Work out the finished part from the listing and answer in its coordinate system (mm). Face numbers are marked on the shaded views. Round coordinates to 2 decimals unless told otherwise and drop trailing zeros. Loops run counter-clockwise (first coordinate to the right, second up) from the corner with the lowest first, then second, coordinate; pieces in that order, holes last. Notation, with made-up numbers: (56, 69) - (106, 69) arc R15 cw to (106, 83) - close; hole circle Ø5 at (12, 31.5). An arc over 180 degrees is marked (long way). Answer as CSV lines item,"result". Start each with the question number.
Q1. Each of these flat-tipped pins is pushed along its axis until it touches: pin 1 Ø5 at (y, z) = (53, 30.5) entering from +X; pin 2 Ø1 at (x, y) = (16.5, 42) entering from +Z; pin 3 Ø3 at (x, z) = (20, 35) entering from +Y; pin 4 Ø3 at (x, z) = (22, -43) entering from -Y. Where does it stop, or does it pass through?
Q2. The mould has two halves that part along Z. Classify the marked faces 1, 2, 3 and 4: +Z half, -Z half, draft (parallel to the pull), parting line (faces both ways), or undercut.
Q3. Straight lines are drawn through the part: L1, parallel to Y at x = 11.25, z = 48.5; L2, parallel to Y at x = 10.25, z = 0; L3, parallel to Y at x = 18.75, z = 48.5. For each, find the intervals that lie inside material, in ascending order. Write a range as [from, to].
Q4. Section B-B on y = 0 is taken. Write down the section's boundary in (x, z).
Q5. Section C-C on x = 19.25 is taken. Write down the section's boundary in (y, z).
Q6. Section D-D on z = 45.5 is taken. Write down the section's boundary in (x, y), then the cut area to 3 significant figures.
Q7. Section A-A on z = 0 is taken. Write down the section's boundary in (x, y), then the cut area to 4 significant figures.
```python
from build123d import *

# Parameters (mm, degrees)
EXTRUDE_1_DEPTH     = 75
SKETCH_2_R          = 30
CUT_EXTRUDE_1_DEPTH = 210
HOLE_WIZARD_M12_1_D = 10.2


with BuildPart() as part:
    # 草图1 → 凸台-拉伸1 (new, symmetric)
    with BuildSketch(Plane.XY):
        Polygon((0, 57.5), (0, -57.5), (15, -57.5), (15, -40.5), (25, -40.5), (25, 40.5), (15, 40.5), (15, 57.5), align=None)
    extrude(amount=EXTRUDE_1_DEPTH, both=True)

    # 草图2 → 切除-拉伸1 (cut)
    with BuildSketch(Plane.ZY):
        Circle(SKETCH_2_R)
    extrude(amount=-CUT_EXTRUDE_1_DEPTH, mode=Mode.SUBTRACT)

    # M12 螺纹孔1 (through all)
    with Locations(Plane.ZY):
        with Locations((-58.5, 30), (48.5, 30), (48.5, -30), (-58.5, -30)):
            Hole(HOLE_WIZARD_M12_1_D / 2)


solid = part.part
```
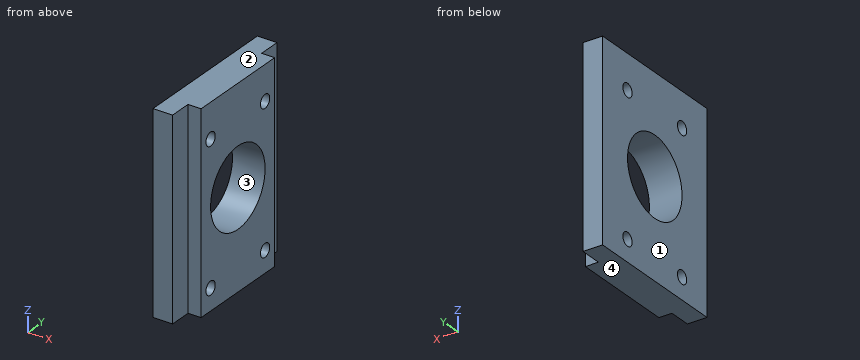
Findings:
1,pin 1,"stops at x = 15"
1,pin 2,"passes through"
1,pin 3,"stops at y = 40.5"
1,pin 4,"stops at y = -40.5"
2,face 1,"draft"
2,face 2,"+Z half"
2,face 3,"undercut"
2,face 4,"-Z half"
3,L1,"y = [-57.5, -35.1], [-24.9, 24.9], [35.1, 57.5]"
3,L2,"y = [-57.5, -30], [30, 57.5]"
3,L3,"y = [-40.5, -35.1], [-24.9, 24.9], [35.1, 40.5]"
4,outline,"(0, -75) - (25, -75) - (25, -30) - (0, -30) - close; (0, 30) - (25, 30) - (25, 75) - (0, 75) - close"
5,outline,"(-40.5, -75) - (40.5, -75) - (40.5, 75) - (-40.5, 75) - close; hole circle Ø10.2 at (-30, -58.5); hole circle Ø10.2 at (-30, 48.5); hole circle Ø60 at (0, 0); hole circle Ø10.2 at (30, -58.5); hole circle Ø10.2 at (30, 48.5)"
6,outline,"(0, -57.5) - (15, -57.5) - (15, -40.5) - (25, -40.5) - (25, -34.12) - (0, -34.12) - close; (0, -25.88) - (25, -25.88) - (25, 25.88) - (0, 25.88) - close; (0, 34.12) - (25, 34.12) - (25, 40.5) - (15, 40.5) - (15, 57.5) - (0, 57.5) - close"
6,area,"2,120 mm^2"
7,outline,"(0, -57.5) - (15, -57.5) - (15, -40.5) - (25, -40.5) - (25, -30) - (0, -30) - close; (0, 30) - (25, 30) - (25, 40.5) - (15, 40.5) - (15, 57.5) - (0, 57.5) - close"
7,area,"1,035 mm^2"
